Read the model definition and answer for the solid it produces. Units are mm, in the model's axes. A direction names the side the tool comes from. Give positions to 0.01 mm unless a question says otherwise; leave off trailing zeros. Order: outer loops, then holes, each group sorted by start corner. A loop starts at its lowest first (then second) coordinate and runs counter-clockwise, first axis right, second up. Notation, with made-up numbers: (70, -33) - (125, -33) arc R15 cw to (125, -17) - close; hole circle Ø2 at (-33, -17.75). An arc over 180 degrees is marked (long way). Write each question's results on one line, items separated by ' | '.
from build123d import *

# Parameters (mm, degrees)
CUT_REVOLVE_1_ANGLE    = 90
CHAMFER_1_SIZE         = 0.5
HOLE_WIZARD_M4_1_D     = 3.3
HOLE_WIZARD_M4_1_DEPTH = 11.5
HOLE_WIZARD_M4_1_TIP   = 0.991420021


with BuildPart() as part:
    # 草图1 → 旋转1 (revolve)
    with BuildSketch(Plane.XY, mode=Mode.PRIVATE) as revolve_1_sk:
        Polygon((0, 30), (10, 30), (10, 20), (107, 20), (107, 28), (99, 28), (99, 28.444863729), (82, 33), (70, 33), (70, 28), (63, 28), (63, 28.444863729), (46, 33), (0, 33), align=None)
    revolve(revolve_1_sk.sketch.rotate(Axis((0, 0, 0), (1, 0, 0)), 90), axis=Axis((0, 0, 0), (1, 0, 0)))

    # 草图2 → 切除-旋转1 (revolve, symmetric, cut)
    with BuildSketch(Plane.XY) as cut_revolve_1_sk:
        Polygon((18, 33), (52.5, 33), (52.5, 38), (102.5, 38), (102.5, 20), (18, 20), align=None)
    cut_revolve_1 = revolve(axis=Axis((0, 0, 0), (1, 0, 0)), revolution_arc=CUT_REVOLVE_1_ANGLE / 2, mode=Mode.SUBTRACT)
    cut_revolve_1 = cut_revolve_1 + revolve(cut_revolve_1_sk.sketch, axis=Axis((0, 0, 0), (-1, 0, 0)), revolution_arc=CUT_REVOLVE_1_ANGLE / 2, mode=Mode.SUBTRACT)

    # 镜向1: 切除-旋转1 across plane
    add(cut_revolve_1.mirror(Plane.ZX), mode=Mode.SUBTRACT)

    # 倒角1
    chamfer_1_edges = [part.edges().sort_by_distance(p)[0] for p in [
        (0, 0, -33),
    ]]
    chamfer(chamfer_1_edges, length=CHAMFER_1_SIZE)

    # M4 螺纹孔1
    with Locations(Plane.ZY.offset(-10)):
        with Locations((0, 25), (25, 0), (0, -25), (-25, 0)):
            Hole(HOLE_WIZARD_M4_1_D / 2, depth=HOLE_WIZARD_M4_1_DEPTH)
            with Locations((0, 0, -(HOLE_WIZARD_M4_1_DEPTH + HOLE_WIZARD_M4_1_TIP / 2))):  # 118° drill point
                Cone(0, HOLE_WIZARD_M4_1_D / 2, HOLE_WIZARD_M4_1_TIP, mode=Mode.SUBTRACT)


solid = part.part
(1) For faces 4 (the face through (102.5, 21, 0)), 5 (the face through (66, 0, 28)), 6 (the face through (14.056, -23.364, 0.215)), 7 (the face through (102.5, -21, 0)), determine the directions among +Z, -Z, +X, -X, +Y, -Y from which every point of the face is accessible in a straight line to the end or side of a thin tool.
Conclusion:
face 4: +Y | face 5: +Z | face 6: -X | face 7: -Y
(2) The mould has two halves that part along Y. Classify faces 1 (the face through (5.07, -25.296, 16.128)), 2 (the face through (76, 0, -33)), 3 (the face through (18, 22, 0)): pulls with the +Y half, pulls with the -Y half, needs draft (parallel to the pull), parting line crosses it, or undercut.
Conclusion:
face 1: undercut | face 2: parting line crosses it | face 3: needs draft
(3) Section A-A (x = 20) is taken. Give the vertices of the cut face in (y, z), plus the area to 3 significant figures.
Conclusion:
outline: (-23.33, -23.33) arc R33 ccw to (23.33, -23.33) - (14.14, -14.14) arc R20 cw to (-14.14, -14.14) - close; (-23.33, 23.33) - (-14.14, 14.14) arc R20 cw to (14.14, 14.14) - (23.33, 23.33) arc R33 ccw to start; hole circle Ø3.3 at (0, -25); hole circle Ø3.3 at (0, 25) | area: 1,070 mm^2
(4) Section B-B (z = 0) is taken. State how many separate pieces and enclosed holes the cut face has, plus the area to 3 significant figures.
Conclusion:
separate pieces: 6 | enclosed holes: 0 | area: 287 mm^2
(5) Section C-C (x = 40) is taken. Give the vertices of the cut face in (y, z), plus the area to 3 significant figures.
Conclusion:
outline: (-23.33, -23.33) arc R33 ccw to (23.33, -23.33) - (14.14, -14.14) arc R20 cw to (-14.14, -14.14) - close; (-23.33, 23.33) - (-14.14, 14.14) arc R20 cw to (14.14, 14.14) - (23.33, 23.33) arc R33 ccw to start | area: 1,080 mm^2
(6) Consider probe 1 along Y at (x, z) = (15, 0); probe 2 along Z at (x, y) = (30, 0.5); probe 3 along X at (y, z) = (-18, -9.5). Determine where each line is inside the solid, lowest interval first. Write a range as [from, to].
Conclusion:
probe 1: [-33, -26.65], [-23.35, -20], [20, 23.35], [26.65, 33] | probe 2: [-33, -19.99], [19.99, 33] | probe 3: [10, 18], [102.5, 107]
(7) Each of these flat-tipped pins is pushed along its axis until it touches: pin 1 (8 mm diameter, centred on x = 83, z = -10.5, fed in from +Y); pin 2 (8 mm diameter, centred on x = 45, y = 8, fed in from +Z); pin 3 (12 mm diameter, centred on x = 77, z = 9, fed in from +Y); pin 4 (14.5 mm diameter, centred on y = -5, z = -28, fed in from -X). Where does it stop, or does it pass through?
Conclusion:
pin 1: y = 14.5 | pin 2: z = 32.76 | pin 3: y = 15 | pin 4: x = 0
